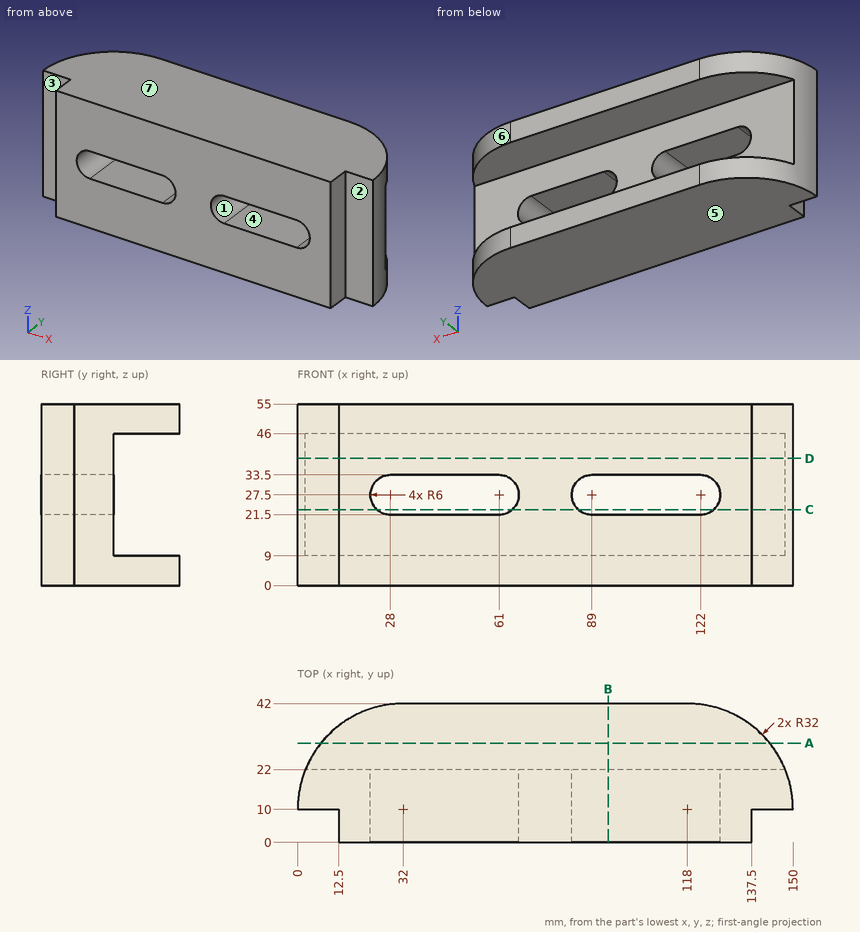
The figure shows three views and two pictorial views of one solid part (mm, origin at its lowest corner). Answer the questions. A direction names the side the tool comes from. Round coordinates to 2 decimals unless told otherwise and drop trailing zeros. Write each loop counter-clockwise with the first axis right and the second up, starting at its lowest first coordinate (ties: lowest second). Pieces come first, ordered by that corner, then holes. Notation, with made-up numbers: M 15,-32.5 L 31,-32.5 A15 cw 31,-27.5 Z; hole C -28,51.25 d6. An arc over 180 degrees is marked long. Use a Markdown table: item, result.
1) Consider line 1 (Z direction, x = 44, y = 38.5); line 2 (Y direction, x = 140, z = 17); line 3 (X direction, y = 7.5, z = 24.5). Determine where each line is inside the solid, lowest interval first. Write a range as [from, to].
Taken from the geometry:
| item | result |
|---|---|
| line 1 | z = [0, 9], [46, 55] |
| line 2 | y = [10, 22] |
| line 3 | x = [12.5, 22.8], [66.2, 83.8], [127.2, 137.5] |
2) Determine the mould class of the marked faces 4, 5, 6 and 7 for opening direction Z: pulls with the +Z half, pulls with the -Z half, needs draft (parallel to the pull), parting line crosses it, or undercut.
Taken from the geometry:
| item | result |
|---|---|
| face 4 | undercut |
| face 5 | pulls with the -Z half |
| face 6 | needs draft |
| face 7 | pulls with the +Z half |
3) Which of the six approach directions +Z, -Z, +X, -X, +Y, -Y give full straight-line access (tool end or side, diameter ignored) to the marked faces 1, 2 and 3?
Taken from the geometry:
| item | result |
|---|---|
| face 1 | +Y, -Y |
| face 2 | +Z, -Z, +X, -Y |
| face 3 | +Z, -Z, -X, -Y |
4) The part is cut by section A-A on y = 30. Give the vertices of the cut face in (x, z).
Taken from the geometry:
| item | result |
|---|---|
| outline | M 7.02,0 L 142.98,0 L 142.98,9 L 7.02,9 Z; M 7.02,46 L 142.98,46 L 142.98,55 L 7.02,55 Z |
5) The part is cut by section D-D on z = 38.5. Give the vertices of the cut face in (x, y), plus the area to 3 significant figures.
Taken from the geometry:
| item | result |
|---|---|
| outline | M 0,10 L 12.5,10 L 12.5,0 L 137.5,0 L 137.5,10 L 150,10 A32 ccw 147.66,22 L 2.34,22 A32 ccw Z |
| area | 3,030 mm2 |
6) The part is cut by section C-C on z = 23. Give the vertices of the cut face in (x, y), plus the area to 3 significant figures.
Taken from the geometry:
| item | result |
|---|---|
| outline | M 0,10 L 12.5,10 L 12.5,0 L 24.03,0 L 24.03,22 L 2.34,22 A32 ccw Z; M 64.97,0 L 85.03,0 L 85.03,22 L 64.97,22 Z; M 125.97,0 L 137.5,0 L 137.5,10 L 150,10 A32 ccw 147.66,22 L 125.97,22 Z |
| area | 1,230 mm2 |
7) The part is cut by section B-B on x = 94. Give the vertices of the cut face in (y, z).
Taken from the geometry:
| item | result |
|---|---|
| outline | M 0,0 L 42,0 L 42,9 L 22,9 L 22,21.5 L 0,21.5 Z; M 0,33.5 L 22,33.5 L 22,46 L 42,46 L 42,55 L 0,55 Z |
8) Flat-ended cylindrical pins translate along their axes: pin 1 (4 mm diameter, centred on y = 12.5, z = 17.5, fed in from +X); pin 2 (1.5 mm diameter, centred on y = 23, z = 7, fed in from -X); pin 3 (3 mm diameter, centred on y = 13.5, z = 44.5, fed in from +X). Find the tip coordinate at first contact, or state that the pin passes through.
Taken from the geometry:
| item | result |
|---|---|
| pin 1 | stops at x = 150 |
| pin 2 | stops at x = 2.44 |
| pin 3 | stops at x = 149.94 |
